Source: CAD feature listing. Evaluate the final solid. Frame: model axes, mm. A direction names the side the tool comes from. Give positions to 0.01 mm unless a question says otherwise; leave off trailing zeros. Loops run counter-clockwise (first coordinate to the right, second up) from the corner with the lowest first, then second, coordinate; pieces in that order, holes last. Notation, with made-up numbers: (-35, -26.5) - (-9, -26.5) arc R20 cw to (-9, 6.5) - close; hole circle Ø1 at (33.5, -33). An arc over 180 degrees is marked (long way). Put each result on its own line as item: value.
```python
from build123d import *

# Parameters (mm, degrees)
SKETCH2_W          = 82.566044685
SKETCH2_H          = 15.592809798
SKETCH2_W_2        = 148.96712198
SKETCH2_H_2        = 11.958140401
CUT_EXTRUDE1_DEPTH = 5


with BuildPart() as part:
    # Sketch1 → Revolve1 (revolve)
    with BuildSketch(Plane.XY, mode=Mode.PRIVATE) as revolve1_sk:
        Polygon((-74.14259961, 26.024332396), (-74.14259961, 17.45458405), (-79.306985444, 17.45458405), (-79.306985444, 6.508165042), (-108, 6.508165042), (-108, 13.551665989), (-109.954236571, 13.551665989), (-111.789002112, 13.551665989), (-111.789002112, 4), (-106.267464057, 4), (-77, 4), (-77, 14.153673902), (-71.527344849, 14.153673902), (-71.527344849, 26.024332396), align=None)
    revolve(revolve1_sk.sketch.rotate(Axis((0, 0, 0), (-1, 0, 0)), 90), axis=Axis((0, 0, 0), (-1, 0, 0)))

    # Sketch2 → Cut-Extrude1 (cut)
    with BuildSketch(Plane.ZY.offset(111.789002112)):
        with Locations((-3.321091868, 13.796404899)):
            Rectangle(SKETCH2_W, SKETCH2_H)
        with Locations((5.512682346, -11.979070201)):
            Rectangle(SKETCH2_W_2, SKETCH2_H_2)
    extrude(amount=-CUT_EXTRUDE1_DEPTH, mode=Mode.SUBTRACT)


solid = part.part
```
1) Section query A-A, the plane z = 0. Output: boundary loops of the cut face in (x, y).
Check result:
outline: (-111.79, -6) - (-106.79, -6) - (-106.79, -6.51) - (-79.31, -6.51) - (-79.31, -17.45) - (-74.14, -17.45) - (-74.14, -26.02) - (-71.53, -26.02) - (-71.53, -14.15) - (-77, -14.15) - (-77, -4) - (-111.79, -4) - close; (-111.79, 4) - (-77, 4) - (-77, 14.15) - (-71.53, 14.15) - (-71.53, 26.02) - (-74.14, 26.02) - (-74.14, 17.45) - (-79.31, 17.45) - (-79.31, 6.51) - (-106.79, 6.51) - (-106.79, 6) - (-111.79, 6) - close
2) Material intervals for line 1 along Y through (x, z) = (-74.05, 0); line 2 along Y through (x, z) = (-104, 0); line 3 along X through (y, z) = (18, -14), sorted ascending. Write a range as [from, to].
Check result:
line 1: [-26.02, -14.15], [14.15, 26.02]
line 2: [-6.51, -4], [4, 6.51]
line 3: [-74.14, -71.53]
3) Mould query, pull axis Y, two halves, no side actions, for faces 1 (the cylindrical face through (-72.853, 25.405, 5.642)), 2 (the flat face through (-110, 6, 0)), 3 (the cylindrical face through (-94.151, 3.905, 0.867)). Classes: pulls with the +Y half, pulls with the -Y half, needs draft (parallel to the pull), parting line crosses it, or undercut.
Check result:
face 1: parting line crosses it
face 2: pulls with the +Y half
face 3: undercut
4) Section query B-B, the plane y = 0. Output: boundary loops of the cut face in (x, z).
Check result:
outline: (-111.79, -13.55) - (-108, -13.55) - (-108, -6.51) - (-79.31, -6.51) - (-79.31, -17.45) - (-74.14, -17.45) - (-74.14, -26.02) - (-71.53, -26.02) - (-71.53, -14.15) - (-77, -14.15) - (-77, -4) - (-111.79, -4) - close; (-111.79, 4) - (-77, 4) - (-77, 14.15) - (-71.53, 14.15) - (-71.53, 26.02) - (-74.14, 26.02) - (-74.14, 17.45) - (-79.31, 17.45) - (-79.31, 6.51) - (-108, 6.51) - (-108, 13.55) - (-111.79, 13.55) - close
5) Access query for faces 4 (the cylindrical face through (-109.92, 0.09, -13.55)), 5 (the cylindrical face through (-74.23, -4.25, -13.5)), 6 (the flat face through (-79.307, 0, -8)), 7 (the cylindrical face through (-109.92, -0.09, 13.55)). Directions: +Z, -Z, +X, -X, +Y, -Y. A direction counts if a zero-diameter tool reaches every point of the face in a straight line with its end or side. Return the directions, or none.
Check result:
face 4: -Z, -X
face 5: +X
face 6: none
face 7: +Z, -X
6) Section query D-D, the plane y = 8.5. Output: boundary loops of the cut face in (x, z), plus the area to 3 significant figures.
Check result:
outline: (-79.31, -15.25) - (-74.14, -15.25) - (-74.14, -24.6) - (-71.53, -24.6) - (-71.53, -11.32) - (-77, -11.32) - (-77, 11.32) - (-71.53, 11.32) - (-71.53, 24.6) - (-74.14, 24.6) - (-74.14, 15.25) - (-79.31, 15.25) - close
area: 162 mm²
7) Pin query (flat end, axial travel): P1, Ø3.5, axis at y = 1, z = 7, coming from the +X side; P2, Ø5, axis at x = -93.5, y = 7, coming from the -Z side; P3, Ø4, axis at x = -110, z = -5.5, coming from the +Y side; P4, Ø10.5, axis at y = 0, z = 0, coming from the -X side. Return the tip coordinate at first contact, or that it passes through.
Check result:
P1: x = -77
P2: z = -4.7
P3: y = 6
P4: x = -111.79
8) Section query C-C, the plane x = -102.5. Output: boundary loops of the cut face in (y, z), plus the area to 3 significant figures.
Check result:
outline: circle Ø13.02 at (0, 0); hole circle Ø8 at (0, 0)
area: 82.8 mm²
